from build123d import *

# Parameters (mm, degrees)
SKETCH1_W           = 90
SKETCH1_H           = 122
BOSS_EXTRUDE1_DEPTH = 12
SKETCH2_R           = 30
CUT_EXTRUDE1_DEPTH  = 77.746335417
SKETCH3_R           = 40.05
CUT_EXTRUDE2_DEPTH  = 6
M6_TAPPED_HOLE1_D   = 5
CUT_EXTRUDE3_DEPTH  = 77.746335417
FILLET1_R           = 5


with BuildPart() as part:
    # Sketch1 → Boss-Extrude1 (new body)
    with BuildSketch(Plane.XY):
        Rectangle(SKETCH1_W, SKETCH1_H)
    extrude(amount=BOSS_EXTRUDE1_DEPTH)

    # Sketch2 → Cut-Extrude1 (cut, through all)
    with BuildSketch(Plane.XY.offset(12)):
        Circle(SKETCH2_R)
    extrude(amount=-CUT_EXTRUDE1_DEPTH, mode=Mode.SUBTRACT)

    # Sketch3 → Cut-Extrude2 (cut)
    with BuildSketch(Plane.XY.offset(12)):
        Circle(SKETCH3_R)
    extrude(amount=-CUT_EXTRUDE2_DEPTH, mode=Mode.SUBTRACT)

    # M6 Tapped Hole1 (through all)
    with Locations(Plane.XY.offset(12)):
        with Locations((35.355339059, 35.355339059), (-35.355339059, 35.355339059), (-35.355339059, -35.355339059), (35.355339059, -35.355339059)):
            Hole(M6_TAPPED_HOLE1_D / 2)

    # Sketch6 → Cut-Extrude3 (cut, through all)
    with BuildSketch(Plane.XY.offset(12)):
        with BuildLine():
            Line((-38.25, 55.5), (-38.25, 49.5))
            ThreePointArc((-38.25, 49.5), (-35, 46.25), (-31.75, 49.5))
            Line((-31.75, 49.5), (-31.75, 55.5))
            ThreePointArc((-31.75, 55.5), (-35, 58.75), (-38.25, 55.5))
        make_face()
        with BuildLine():
            ThreePointArc((38.25, 49.5), (35, 46.25), (31.75, 49.5))
            Line((31.75, 49.5), (31.75, 55.5))
            ThreePointArc((31.75, 55.5), (35, 58.75), (38.25, 55.5))
            Line((38.25, 55.5), (38.25, 49.5))
        make_face()
        with BuildLine():
            Line((38.25, -55.5), (38.25, -49.5))
            ThreePointArc((38.25, -49.5), (35, -46.25), (31.75, -49.5))
            Line((31.75, -49.5), (31.75, -55.5))
            ThreePointArc((31.75, -55.5), (35, -58.75), (38.25, -55.5))
        make_face()
        with BuildLine():
            ThreePointArc((-38.25, -49.5), (-35, -46.25), (-31.75, -49.5))
            Line((-31.75, -49.5), (-31.75, -55.5))
            ThreePointArc((-31.75, -55.5), (-35, -58.75), (-38.25, -55.5))
            Line((-38.25, -55.5), (-38.25, -49.5))
        make_face()
    extrude(amount=-CUT_EXTRUDE3_DEPTH, mode=Mode.SUBTRACT)

    # Fillet1
    fillet1_edges = [part.edges().sort_by_distance(p)[0] for p in [
        (45, -61, 6),
        (-45, -61, 6),
        (-45, 61, 6),
        (45, 61, 6),
    ]]
    fillet(fillet1_edges, radius=FILLET1_R)


solid = part.part
Geometry check sheet. Reference: the model listing, model coordinates, mm. A direction names the side the tool comes from. Coordinates: 2 decimals unless noted, no trailing zeros. Order: outer loops, then holes, each group sorted by start corner. A loop starts at its lowest first (then second) coordinate and runs counter-clockwise, first axis right, second up. Notation, with made-up numbers: (-29.5, 43.25) - (26.5, 43.25) arc R16 cw to (26.5, 63.25) - close; hole circle Ø5 at (29, 43). An arc over 180 degrees is marked (long way). One line per item, written item: value.
(1) Sectioned sample at B-B (x = 0). Enter the section's corners in (y, z).
Data:
outline: (-61, 0) - (-30, 0) - (-30, 6) - (-40.05, 6) - (-40.05, 12) - (-61, 12) - close; (30, 0) - (61, 0) - (61, 12) - (40.05, 12) - (40.05, 6) - (30, 6) - close
(2) Access from +Z, -Z, +X, -X, +Y, -Y to the whole of each face (thin tool, end or side, straight path). Record for faces 5 (the face through (-1, 61, 6)), 6 (the face through (-34.93, -58.75, 6.08)), 7 (the face through (-29.519, 27.068, 9.042)).
Data:
face 5: +Z, -Z, +X, -X, +Y
face 6: +Z, -Z
face 7: +Z
(3) Thickness scan on probe 1 along Y at (x, z) = (0, 8.05); probe 2 along Y at (x, z) = (0, 3.3); probe 3 along Z at (x, y) = (14.5, -36). Record the ranges inside material, lowest first. Write a range as from..to.
Data:
probe 1: y = -61..-40.05, 40.05..61
probe 2: y = -61..-30, 30..61
probe 3: z = 0..6
(4) Release check for a two-part mould opening along Y. For faces 1 (the face through (31.75, 52, 6)), 2 (the face through (43, -60, 6)), 3 (the face through (43, 60, 6)), 4 (the face through (33.046, -36.313, 5.916)) record: +Y half, -Y half, draft (parallel to the pull), parting line (faces both ways), or undercut.
Data:
face 1: undercut
face 2: -Y half
face 3: +Y half
face 4: undercut
(5) Sectioned sample at A-A (y = 52). Enter the section's corners in (x, z).
Data:
outline: (-45, 0) - (-38.25, 0) - (-38.25, 12) - (-45, 12) - close; (-31.75, 0) - (31.75, 0) - (31.75, 12) - (-31.75, 12) - close; (38.25, 0) - (45, 0) - (45, 12) - (38.25, 12) - close
(6) Sectioned sample at C-C (y = 0). Enter the section's corners in (x, z), and give its area (3 significant figures).
Data:
outline: (-45, 0) - (-30, 0) - (-30, 6) - (-40.05, 6) - (-40.05, 12) - (-45, 12) - close; (30, 0) - (45, 0) - (45, 12) - (40.05, 12) - (40.05, 6) - (30, 6) - close
area: 239 mm^2
(7) Sectioned sample at D-D (x = -35). Enter the section's corners in (y, z).
Data:
outline: (-61, 0) - (-58.75, 0) - (-58.75, 12) - (-61, 12) - close; (-46.25, 0) - (-37.83, 0) - (-37.83, 12) - (-46.25, 12) - close; (-32.88, 0) - (32.88, 0) - (32.88, 12) - (19.47, 12) - (19.47, 6) - (-19.47, 6) - (-19.47, 12) - (-32.88, 12) - close; (37.83, 0) - (46.25, 0) - (46.25, 12) - (37.83, 12) - close; (58.75, 0) - (61, 0) - (61, 12) - (58.75, 12) - close
